For this review, take the finished solid that the model builds, in its own axes (mm). Coordinates: 2 decimals unless noted, no trailing zeros. Loops run counter-clockwise (first coordinate to the right, second up) from the corner with the lowest first, then second, coordinate; pieces in that order, holes last.
```python
from build123d import *

# Parameters (mm, degrees)
BOSS_EXTRUDE1_DEPTH = 480


with BuildPart() as part:
    # Sketch1 → Boss-Extrude1 (new body)
    with BuildSketch(Plane.XY):
        Polygon((5, 5), (5, 10), (15, 10), (15, 5), (20, 5), (20, 0), (0, 0), (0, 5), align=None)
    extrude(amount=BOSS_EXTRUDE1_DEPTH)


solid = part.part
```
Q1. For pin 1 Ø6 at (x, y) = (13.5, 4) entering from -Z; pin 2 Ø2.5 at (x, z) = (16.5, 252.5) entering from +Y; pin 3 Ø1 at (y, z) = (7, 312.5) entering from +X; pin 4 Ø4 at (y, z) = (8.5, 134) entering from -X, all flat-tipped, find the tip position at first contact; note any pin that passes through.
Q2. Wall thickness on probe 1 along X at (y, z) = (8.5, 364.5); probe 2 along Y at (x, z) = (16.5, 213.5): over which ranges is each line inside the solid? List them lowest first.
Q3. Consider section A-A (z = 254). State the section outline as (x, y) points.
Q4. Consider section B-B (y = 7.5). State the section outline as (x, z) points, then the cut area to 3 significant figures.
Model answer:
1. pin 1: stops at z = 0
1. pin 2: stops at y = 5
1. pin 3: stops at x = 15
1. pin 4: stops at x = 5
2. probe 1: x = 5 to 15
2. probe 2: y = 0 to 5
3. outline: (0, 0) - (20, 0) - (20, 5) - (15, 5) - (15, 10) - (5, 10) - (5, 5) - (0, 5) - close
4. outline: (5, 0) - (15, 0) - (15, 480) - (5, 480) - close
4. area: 4,800 mm2
